Geometry: final body of the model. Coordinates: model frame, mm. Face numbers are marked on the shaded views. Give positions to 0.01 mm unless a question says otherwise; leave off trailing zeros. Write each loop counter-clockwise with the first axis right and the second up, starting at its lowest first coordinate (ties: lowest second). Pieces come first, ordered by that corner, then holes. Notation, with made-up numbers: (-16.75, 69) -> (-6.75, 69) arc R17 cw to (-6.75, 86) -> close; hole circle Ø10 at (49.25, 80). An arc over 180 degrees is marked (long way). Answer as a JSON object with one key per item and string values. Group by question number.
(1) Draft query along Y for the marked faces 1, 2 and 3. Return one class per face: +Y half, -Y half, draft (parallel to the pull), parting line (faces both ways), or undercut.
(2) Contact query for flat-ended pins moving along their axis: pin 1 Ø5.5 at (x, y) = (3.5, -4.5) entering from -Z; pin 2 Ø1 at (y, z) = (-4.5, -76.5) entering from -X; pin 3 Ø3 at (y, z) = (5, -16) entering from -X. Output: stop coordinate, or through.
(3) Material intervals for probe 1 along X at (y, z) = (0, -3); probe 2 along X at (y, z) = (-0.25, -104), sorted ascending.
(4) Section query B-B on z = -75.5. Output: boundary loops of the cut face in (x, y), plus the area to 3 significant figures.
(5) Section query C-C on z = -7. Output: boundary loops of the cut face in (x, y).
(6) Section query D-D on z = -43.5. Output: boundary loops of the cut face in (x, y), plus the area to 3 significant figures.
(7) Section query A-A on x = 0. Output: boundary loops of the cut face in (y, z).
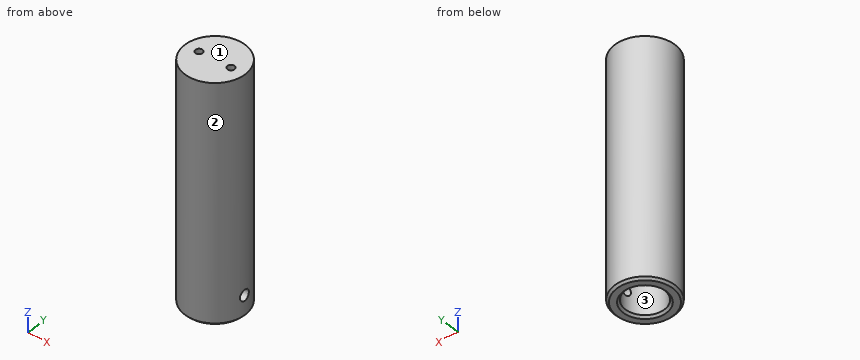
from build123d import *

# Parameters (mm, degrees)
M4_TAPPED_HOLE1_D     = 3.3
M4_TAPPED_HOLE1_DEPTH = 10.1
M4_TAPPED_HOLE1_TIP   = 0.991420021
M6_TAPPED_HOLE1_D     = 5
M6_TAPPED_HOLE1_DEPTH = 17
M6_TAPPED_HOLE1_TIP   = 1.502151548
CHAMFER1_SIZE         = 1


with BuildPart() as part:
    # Sketch1 → Revolve1 (revolve)
    with BuildSketch(Plane(origin=(0, 0, 0), x_dir=(1, 0, 0), z_dir=(0, 1, 0))):
        Polygon((-9.05, 110), (-14, 110), (-14, 0), (0, 0), (0, 50), (-9.05, 50), align=None)
    revolve(axis=Axis((0, 0, -50), (0, 0, 1)))

    # M4 Tapped Hole1
    with Locations(Plane(origin=(-7.5, 0, 0), x_dir=(1, 0, 0), z_dir=(0, 0, 1))):
        with Locations((0, 0), (15, 0)):
            Hole(M4_TAPPED_HOLE1_D / 2, depth=M4_TAPPED_HOLE1_DEPTH)
            with Locations((0, 0, -(M4_TAPPED_HOLE1_DEPTH + M4_TAPPED_HOLE1_TIP / 2))):  # 118° drill point
                Cone(0, M4_TAPPED_HOLE1_D / 2, M4_TAPPED_HOLE1_TIP, mode=Mode.SUBTRACT)

    # M6 Tapped Hole1
    with Locations(Plane(origin=(14, 0, -100), x_dir=(0, 1, 0), z_dir=(1, 0, 0))):
        with Locations((0, 0)):
            Hole(M6_TAPPED_HOLE1_D / 2, depth=M6_TAPPED_HOLE1_DEPTH)
            with Locations((0, 0, -(M6_TAPPED_HOLE1_DEPTH + M6_TAPPED_HOLE1_TIP / 2))):  # 118° drill point
                Cone(0, M6_TAPPED_HOLE1_D / 2, M6_TAPPED_HOLE1_TIP, mode=Mode.SUBTRACT)

    # Chamfer1
    chamfer1_edges = [part.edges().sort_by_distance(p)[0] for p in [
        (14, 0, -110),
        (9.05, 0, -110),
    ]]
    chamfer(chamfer1_edges, length=CHAMFER1_SIZE)


solid = part.part
Answer list:
{
 "1": {"face 1": "draft", "face 2": "parting line", "face 3": "undercut"},
 "2": {"pin 1": "z = -50", "pin 2": "x = -13.42", "pin 3": "x = -13.56"},
 "3": {"probe 1": "-14 to -9.15, -5.85 to 5.85, 9.15 to 14", "probe 2": "-14 to -9.05, 9.05 to 14"},
 "4": {"outline": "circle Ø28 at (0, 0); hole circle Ø18.1 at (0, 0)", "area": "358 mm2"},
 "5": {"outline": "circle Ø28 at (0, 0); hole circle Ø3.3 at (-7.5, 0); hole circle Ø3.3 at (7.5, 0)"},
 "6": {"outline": "circle Ø28 at (0, 0)", "area": "616 mm2"},
 "7": {"outline": "(-14, -109) -> (-13, -110) -> (-10.05, -110) -> (-9.05, -109) -> (-9.05, -50) -> (9.05, -50) -> (9.05, -109) -> (10.05, -110) -> (13, -110) -> (14, -109) -> (14, 0) -> (-14, 0) -> close"}
}
